from build123d import *

# Parameters (mm, degrees)
SKETCH1_R           = 8.647
SKETCH1_R_2         = 13
SKETCH1_R_3         = 10.376
SKETCH1_R_4         = 25
BOSS_EXTRUDE1_DEPTH = 40
SKETCH2_R           = 20
CUT_EXTRUDE1_DEPTH  = 25


with BuildPart() as part:
    # Sketch1 → Boss-Extrude1 (new body)
    with BuildSketch(Plane.XY):
        Polygon((498.749353033, 365), (-361.250646967, 365), (-371.250646967, 355), (-371.250646967, -505), (-361.250646967, -515), (498.749353033, -515), (508.749353033, -505), (508.749353033, 355), align=None)
        with Locations((428.749353033, -435)):
            Circle(SKETCH1_R, mode=Mode.SUBTRACT)
        with Locations((-291.250646967, 285)):
            Circle(SKETCH1_R, mode=Mode.SUBTRACT)
        with Locations((428.749353033, 285)):
            Circle(SKETCH1_R, mode=Mode.SUBTRACT)
        with Locations((-291.250646967, -435)):
            Circle(SKETCH1_R, mode=Mode.SUBTRACT)
        with Locations((484.749353033, -491)):
            Circle(SKETCH1_R_2, mode=Mode.SUBTRACT)
        with Locations((-347.250646967, 341)):
            Circle(SKETCH1_R_2, mode=Mode.SUBTRACT)
        with Locations((484.749353033, 341)):
            Circle(SKETCH1_R_2, mode=Mode.SUBTRACT)
        with Locations((-347.250646967, -491)):
            Circle(SKETCH1_R_2, mode=Mode.SUBTRACT)
        with Locations((-107.250646967, -101)):
            Circle(SKETCH1_R_3, mode=Mode.SUBTRACT)
        with Locations((94.749353033, 101)):
            Circle(SKETCH1_R_3, mode=Mode.SUBTRACT)
        with Locations((-107.250646967, 101)):
            Circle(SKETCH1_R_3, mode=Mode.SUBTRACT)
        with Locations((94.749353033, -101)):
            Circle(SKETCH1_R_3, mode=Mode.SUBTRACT)
        with Locations((-246.250646967, -240)):
            Circle(SKETCH1_R_4, mode=Mode.SUBTRACT)
        with Locations((233.749353033, 240)):
            Circle(SKETCH1_R_4, mode=Mode.SUBTRACT)
        with Locations((-246.250646967, 240)):
            Circle(SKETCH1_R_4, mode=Mode.SUBTRACT)
        with Locations((233.749353033, -240)):
            Circle(SKETCH1_R_4, mode=Mode.SUBTRACT)
    extrude(amount=BOSS_EXTRUDE1_DEPTH)

    # Sketch2 → Cut-Extrude1 (cut)
    with BuildSketch(Plane.XY.offset(40)):
        with Locations((-347.250646967, 341)):
            Circle(SKETCH2_R)
        with Locations((484.749353033, 341)):
            Circle(SKETCH2_R)
        with Locations((484.749353033, -491)):
            Circle(SKETCH2_R)
        with Locations((-347.250646967, -491)):
            Circle(SKETCH2_R)
    extrude(amount=-CUT_EXTRUDE1_DEPTH, mode=Mode.SUBTRACT)


solid = part.part
Check sheet for the modelled part. Datum: model origin and axes. Units: mm. A direction names the side the tool comes from. Give positions to 0.01 mm unless a question says otherwise; leave off trailing zeros. Write each loop counter-clockwise with the first axis right and the second up, starting at its lowest first coordinate (ties: lowest second). Pieces come first, ordered by that corner, then holes. Notation, with made-up numbers: (26.25, -37.5) -> (69.25, -37.5) arc R36 cw to (69.25, 1.5) -> close; hole circle Ø11 at (-25, 15.5). An arc over 180 degrees is marked (long way). One line per item, written item: value. Start each with the question number.
Item 1: Section check D-D on y = -101. Record the cut outline in (x, z).
Item 2: Tool access check on faces 1 (the cylindrical face through (490.75, -502.53, 7.4)), 2 (the cylindrical face through (503.224, -498.66, 27.675)). Record the directions out of +Z, -Z, +X, -X, +Y, -Y that give a thin tool (end or side, any length) a straight path to the whole face; none if there is none.
Item 3: Material ranges on probe 1 along X at (y, z) = (-491, 8); probe 2 along Y at (x, z) = (-103.5, 35); probe 3 along Y at (x, z) = (-331, 38), recorded low to high. Write a range as from..to.
Item 4: Section check A-A on y = 240. Record the cut outline in (x, z).
Item 5: Gauge pin test, flat end, axial feed: pin 1 (16.5 mm diameter, centred on x = -107.25, y = 101, fed in from -Z). Record the tip position at first contact, or that the pin passes through.
Item 6: Draft check along Y on faces 3 (the flat face through (508.749, -81, 20)), 4 (the cylindrical face through (247.19, -218.92, 19.72)), 5 (the flat face through (75, 365, 20)). Enter one of: +Y half, -Y half, draft (parallel to the pull), parting line (faces both ways), or undercut.
Item 7: Section check B-B on z = 8.5. State how many separate pieces and enclosed holes the cut face has, then the cut area to 3 significant figures.
Item 8: Section check C-C on y = 341. Record the cut outline in (x, z), then the cut area to 3 significant figures.
Results list:
1. outline: (-371.25, 0) -> (-117.63, 0) -> (-117.63, 40) -> (-371.25, 40) -> close; (-96.87, 0) -> (84.37, 0) -> (84.37, 40) -> (-96.87, 40) -> close; (105.13, 0) -> (508.75, 0) -> (508.75, 40) -> (105.13, 40) -> close
2. face 1: +Z, -Z
2. face 2: +Z
3. probe 1: -371.25..-360.25, -334.25..471.75, 497.75..508.75
3. probe 2: -515..-110.67, -91.33..91.33, 110.67..365
3. probe 3: -515..-502.66, -479.34..329.34, 352.66..365
4. outline: (-371.25, 0) -> (-271.25, 0) -> (-271.25, 40) -> (-371.25, 40) -> close; (-221.25, 0) -> (208.75, 0) -> (208.75, 40) -> (-221.25, 40) -> close; (258.75, 0) -> (508.75, 0) -> (508.75, 40) -> (258.75, 40) -> close
5. pin 1: through
6. face 3: draft
6. face 4: undercut
6. face 5: +Y half
7. separate pieces: 1
7. enclosed holes: 16
7. area: 762,000 mm²
8. outline: (-371.25, 0) -> (-360.25, 0) -> (-360.25, 15) -> (-367.25, 15) -> (-367.25, 40) -> (-371.25, 40) -> close; (-334.25, 0) -> (471.75, 0) -> (471.75, 15) -> (464.75, 15) -> (464.75, 40) -> (-327.25, 40) -> (-327.25, 15) -> (-334.25, 15) -> close; (497.75, 0) -> (508.75, 0) -> (508.75, 40) -> (504.75, 40) -> (504.75, 15) -> (497.75, 15) -> close
8. area: 32,400 mm²
